Geometry check sheet. Reference: the model listing, model coordinates, mm. A direction names the side the tool comes from. Give positions to 0.01 mm unless a question says otherwise; leave off trailing zeros. Write each loop counter-clockwise with the first axis right and the second up, starting at its lowest first coordinate (ties: lowest second). Pieces come first, ordered by that corner, then holes.
(1) Tool access check on faces 4 (the cylindrical face through (54.49, -7.1, 10.9)), 5 (the flat face through (26, -12, 2)). Record the directions out of +Z, -Z, +X, -X, +Y, -Y that give a thin tool (end or side, any length) a straight path to the whole face; none if there is none.
(2) Cross-section at A-A (y = 0). Record the boundary of the cut face in (x, z), and give its area (3 significant figures).
(3) Cross-section at B-B (x = 36.5). Record the boundary of the cut face in (y, z).
(4) Mould release check, pull along X, two halves, no side actions. Record for faces 1 (the flat face through (26, 0, 0)), 2 (the flat face through (26, 0, 18.5)), 3 (the cylindrical face through (-12, 0, 20)): +X half, -X half, draft (parallel to the pull), parting line (faces both ways), or undercut.
(5) Depth check by flat-ended pin: P1, Ø8, axis at y = 9, z = 9.5, coming from the +X side (3 decimals); P2, Ø3, axis at x = 46, z = 13.5, coming from the -Y side; P3, Ø2, axis at x = 1.5, z = 11.5, coming from the +Y side. Enter the tip coordinate at first touch or a pass-through.
(6) Cross-section at D-D (y = -6.75). Record the boundary of the cut face in (x, z), and give its area (3 significant figures).
(7) Cross-section at C-C (z = 10). Record the boundary of the cut face in (x, y).
(8) Thickness scan on line 1 along Y through (x, z) = (0, 6.5); line 2 along Z through (x, y) = (11.5, -5.25); line 3 along X through (y, z) = (3.5, 21.25). Record the ranges inside material, lowest first.
```python
from build123d import *

# Parameters (mm, degrees)
REAR_LINK_PLATE_DEPTH  = 3.5
ROLLER_PROFILES_R      = 8
ROLLERS_2X_16_DEPTH    = 15
FRONT_LINK_PLATE_DEPTH = 3.5
PIN_BORE_PROFILES_R    = 4
PIN_BORES_2X_8_DEPTH   = 22


with BuildPart() as part:
    # Rear Plate Profile → Rear Link Plate (new body)
    with BuildSketch(Plane.XY):
        with BuildLine():
            Line((0, 12), (50.8, 12))
            ThreePointArc((50.8, 12), (62.8, 0), (50.8, -12))
            Line((50.8, -12), (0, -12))
            ThreePointArc((0, -12), (-12, 0), (0, 12))
        make_face()
    extrude(amount=REAR_LINK_PLATE_DEPTH)

    # Roller Profiles → Rollers 2xØ16 (add)
    with BuildSketch(Plane.XY.offset(3.5)):
        Circle(ROLLER_PROFILES_R)
        with Locations((50.8, 0)):
            Circle(ROLLER_PROFILES_R)
    extrude(amount=ROLLERS_2X_16_DEPTH)

    # Front Plate Profile → Front Link Plate (add)
    with BuildSketch(Plane.XY.offset(18.5)):
        with BuildLine():
            Line((0, 12), (50.8, 12))
            ThreePointArc((50.8, 12), (62.8, 0), (50.8, -12))
            Line((50.8, -12), (0, -12))
            ThreePointArc((0, -12), (-12, 0), (0, 12))
        make_face()
    extrude(amount=FRONT_LINK_PLATE_DEPTH)

    # Pin Bore Profiles → Pin Bores 2xØ8 (cut)
    with BuildSketch(Plane.XY.offset(22)):
        Circle(PIN_BORE_PROFILES_R)
        with Locations((50.8, 0)):
            Circle(PIN_BORE_PROFILES_R)
    extrude(amount=-PIN_BORES_2X_8_DEPTH, mode=Mode.SUBTRACT)


solid = part.part
```
Reply:
1. face 4: none
1. face 5: +Z, -Z, +X, -X, -Y
2. outline: (-12, 0) - (-4, 0) - (-4, 22) - (-12, 22) - (-12, 18.5) - (-8, 18.5) - (-8, 3.5) - (-12, 3.5) - close; (4, 0) - (46.8, 0) - (46.8, 22) - (4, 22) - close; (54.8, 0) - (62.8, 0) - (62.8, 3.5) - (58.8, 3.5) - (58.8, 18.5) - (62.8, 18.5) - (62.8, 22) - (54.8, 22) - close; hole (8, 3.5) - (42.8, 3.5) - (42.8, 18.5) - (8, 18.5) - close
2. area: 652 mm2
3. outline: (-12, 0) - (12, 0) - (12, 3.5) - (-12, 3.5) - close; (-12, 18.5) - (12, 18.5) - (12, 22) - (-12, 22) - close
4. face 1: draft
4. face 2: undercut
4. face 3: -X half
5. P1: stops at x = 57.045
5. P2: stops at y = -7.29
5. P3: stops at y = 7.98
6. outline: (-9.92, 0) - (60.72, 0) - (60.72, 3.5) - (55.09, 3.5) - (55.09, 18.5) - (60.72, 18.5) - (60.72, 22) - (-9.92, 22) - (-9.92, 18.5) - (-4.29, 18.5) - (-4.29, 3.5) - (-9.92, 3.5) - close; hole (4.29, 3.5) - (46.51, 3.5) - (46.51, 18.5) - (4.29, 18.5) - close
6. area: 752 mm2
7. outline: circle Ø16 at (0, 0); circle Ø16 at (50.8, 0); hole circle Ø8 at (0, 0); hole circle Ø8 at (50.8, 0)
8. line 1: y = -8 to -4, 4 to 8
8. line 2: z = 0 to 3.5, 18.5 to 22
8. line 3: x = -11.48 to -1.94, 1.94 to 48.86, 52.74 to 62.28
